Part model, mm, in its own coordinate system. Coordinates: 2 decimals unless noted, no trailing zeros. Write each loop counter-clockwise with the first axis right and the second up, starting at its lowest first coordinate (ties: lowest second). Pieces come first, ordered by that corner, then holes. Notation, with made-up numbers: (19, -28) -> (46, -28) arc R27 cw to (46, -2) -> close; hole circle Ø7 at (26, -39). An arc over 180 degrees is marked (long way). Write item = value, one per line. Start each with the question number.
Q1. Band-saw the part on D-D, the plane y = -125. List the corners of the cut face in (x, z), plus the area to 3 significant figures.
Q2. Band-saw the part on B-B, the plane x = 0. List the corners of the cut face in (y, z), plus the area to 3 significant figures.
Q3. Band-saw the part on C-C, the plane z = 7. List the corners of the cut face in (x, y).
Q4. Pin check, flat tips, straight feed: P1, Ø6, axis at y = 77, z = 5.5, coming from the -X side; P2, Ø2, axis at x = -95.5, z = 12.5, coming from the -Y side; P3, Ø6, axis at y = 56, z = 5, coming from the -X side. Stop position of each tip, or through.
Q5. Band-saw the part on A-A, the plane y = 0. List the corners of the cut face in (x, z), plus the area to 3 significant figures.
Q6. Probe line 1 (X direction, y = -16, z = 16); line 2 (Y direction, x = 0, z = 14.25); line 3 (X direction, y = -15.5, z = 1.25). List the from-to ranges inside material, lowest first.
Q7. Pull direction X, two halves, no side cores. Call faces 1 (the flat face through (214.15, 64.88, 9.86)), 2 (the flat face through (158, 1, 0)), 3 (the cylindrical face through (323.846, 7.509, 9.86)): released by +X, released by -X, zero draft, split by the parting line, or undercut.
from build123d import *

# Parameters (mm, degrees)
SKETCH1_R           = 25
SKETCH1_R_2         = 136.5
BOSS_EXTRUDE1_DEPTH = 20


with BuildPart() as part:
    # Sketch1 → Boss-Extrude1 (new body)
    with BuildSketch(Plane.XY):
        with BuildLine():
            Line((122.728358581, 80), (308.159136141, 49.329793203))
            ThreePointArc((308.159136141, 49.329793203), (350, 0), (308.159136141, -49.329793203))
            Line((308.159136141, -49.329793203), (122.728358581, -80))
            ThreePointArc((122.728358581, -80), (-146.5, 0), (122.728358581, 80))
        make_face()
        with Locations((300, 0)):
            Circle(SKETCH1_R, mode=Mode.SUBTRACT)
        Circle(SKETCH1_R_2, mode=Mode.SUBTRACT)
    extrude(amount=BOSS_EXTRUDE1_DEPTH)


solid = part.part
Ans:
q1.outline = (-76.4, 0) -> (-54.84, 0) -> (-54.84, 20) -> (-76.4, 20) -> close; (54.84, 0) -> (76.4, 0) -> (76.4, 20) -> (54.84, 20) -> close
q1.area = 863 mm2
q2.outline = (-146.5, 0) -> (-136.5, 0) -> (-136.5, 20) -> (-146.5, 20) -> close; (136.5, 0) -> (146.5, 0) -> (146.5, 20) -> (136.5, 20) -> close
q2.area = 400 mm2
q3.outline = (122.73, -80) -> (308.16, -49.33) arc R50 ccw to (308.16, 49.33) -> (122.73, 80) arc R146.5 ccw (long way) to start; hole circle Ø273 at (0, 0); hole circle Ø50 at (300, 0)
q4.P1 = -126.44
q4.P2 = -111.95
q4.P3 = -136.58
q5.outline = (-146.5, 0) -> (-136.5, 0) -> (-136.5, 20) -> (-146.5, 20) -> close; (136.5, 0) -> (275, 0) -> (275, 20) -> (136.5, 20) -> close; (325, 0) -> (350, 0) -> (350, 20) -> (325, 20) -> close
q5.area = 3,470 mm2
q6.line_1 = -145.62 to -135.56, 135.56 to 280.79, 319.21 to 347.37
q6.line_2 = -146.5 to -136.5, 136.5 to 146.5
q6.line_3 = -145.68 to -135.62, 135.62 to 280.38, 319.62 to 347.54
q7.face_1 = released by +X
q7.face_2 = zero draft
q7.face_3 = undercut
